Check sheet for the modelled part. Datum: model origin and axes. Units: mm. A direction names the side the tool comes from. Round coordinates to 2 decimals unless told otherwise and drop trailing zeros. Order: outer loops, then holes, each group sorted by start corner. A loop starts at its lowest first (then second) coordinate and runs counter-clockwise, first axis right, second up. Notation, with made-up numbers: (80, 67.25) -> (117, 67.25) arc R29 cw to (117, 106.25) -> close; hole circle Ø2 at (28.25, 60). An arc over 180 degrees is marked (long way). Answer in a Markdown table with one row per item. Add a question column.
1. Sectioned sample at B-B, the plane z = 0. Record the boundary of the cut face in (x, y) (3 decimals), then the cut area to 3 significant figures.
2. Sectioned sample at C-C, the plane y = 28. Record the boundary of the cut face in (x, z) (3 decimals).
3. Sectioned sample at A-A, the plane y = 3. Count the separate pieces of the cut face and the enclosed holes in it, then the cut area to 3 significant figures.
4. Access from +Z, -Z, +X, -X, +Y, -Y to the whole of each face (thin tool, end or side, straight path). Record for faces 1 (the flat face through (43.4, 11.768, -68.4)), 2 (the flat face through (76, 51.143, 0)), 3 (the flat face through (7.501, 57, 76)), 4 (the flat face through (-1, 11.768, -1)).
5. Material ranges on L1, parallel to Z at x = -6.5, y = 7.5; L2, parallel to X at y = 42.5, z = -4; L3, parallel to X at y = 58.5, z = -48, recorded low to high. Write a range as from..to.
6. Depth check by flat-ended pin: P1, Ø4.5, axis at y = 57, z = -76, coming from the -X side; P2, Ø5, axis at x = -1, z = -75.5, coming from the +Y side; P3, Ø6, axis at x = 37.5, y = 16, coming from the +Z side; P4, Ø9, axis at x = 0, z = 103.12, coming from the -Y side. Enter the tip coordinate at first touch or a pass-through.
7. Draft check along Z on faces 5 (the flat face through (0, 51.143, -76)), 6 (the flat face through (-76, 57, -7.5)), 7 (the cylindrical face through (30.881, 51.936, -74.477)), 8 (the flat face through (-76, 57, 7.5)). Enter one of: +Z half, -Z half, draft (parallel to the pull), parting line (faces both ways), or undercut.
```python
from build123d import *

# Parameters (mm, degrees)
SKETCH3_W          = 31.782249742
SKETCH3_H          = 8
SKETCH3_W_2        = 8
SKETCH3_H_2        = 31.782249742
CUT_EXTRUDE1_DEPTH = 6
CHAMFER1_SIZE      = 2
SKETCH4_R          = 4
CUT_EXTRUDE2_DEPTH = 67
SCALE_1_SCALE      = 1.875


with BuildPart() as part:
    # Sketch2 → Revolve1 (revolve)
    with BuildSketch(Plane.XY, mode=Mode.PRIVATE) as revolve1_sk:
        with BuildLine():
            Line((65, 9), (65, 0))
            Line((65, 0), (31, 0))
            Line((31, 0), (29, 2))
            Line((29, 2), (0, 2))
            Line((0, 2), (0, 11))
            Line((0, 11), (30.347168885, 11))
            ThreePointArc((30.347168885, 11), (33.667283917, 12.261439291), (35.312149528, 15.40926553))
            Line((35.312149528, 15.40926553), (39, 38))
            Line((39, 38), (43, 38))
            Line((43, 38), (43, 27))
            Line((43, 27), (45, 27))
            Line((45, 27), (45, 11))
            Line((45, 11), (43, 11))
            Line((43, 11), (43, 9))
            Line((43, 9), (65, 9))
        make_face()
    revolve(revolve1_sk.sketch.rotate(Axis((0, 2, 0), (0, 1, 0)), 90), axis=Axis((0, 2, 0), (0, 1, 0)))

    # Sketch3 → Cut-Extrude1 (cut)
    with BuildSketch(Plane(origin=(0, 38, 0), x_dir=(1, 0, 0), z_dir=(0, 1, 0))):
        with Locations((40.073271414, 0)):
            Rectangle(SKETCH3_W, SKETCH3_H)
        with Locations((0, 40.073271414)):
            Rectangle(SKETCH3_W_2, SKETCH3_H_2)
        with Locations((0, -40.073271414)):
            Rectangle(SKETCH3_W_2, SKETCH3_H_2)
        with Locations((-40.073271414, 0)):
            Rectangle(SKETCH3_W, SKETCH3_H)
    extrude(amount=-CUT_EXTRUDE1_DEPTH, mode=Mode.SUBTRACT)

    # Chamfer1
    chamfer1_edges = [part.edges().sort_by_distance(p)[0] for p in [
        (0, 0, 65),
    ]]
    chamfer(chamfer1_edges, length=CHAMFER1_SIZE)

    # Sketch4 → Cut-Extrude2 (cut)
    with BuildSketch(Plane(origin=(0, 38, 0), x_dir=(1, 0, 0), z_dir=(0, 1, 0))):
        with Locations(Location((0, 55, 0), (0, 0, 270))):
            Circle(SKETCH4_R)
        with Locations(Location((47.817664455, 27.174822282, 0), (0, 0, 270))):
            Circle(SKETCH4_R)
        with Locations(Location((-47.631397208, 27.5, 0), (0, 0, 270))):
            Circle(SKETCH4_R)
        with Locations(Location((-47.631397208, -27.5, 0), (0, 0, 270))):
            Circle(SKETCH4_R)
        with Locations(Location((0, -55, 0), (0, 0, 270))):
            Circle(SKETCH4_R)
        with Locations(Location((47.817664455, -27.174822282, 0), (0, 0, 270))):
            Circle(SKETCH4_R)
    extrude(amount=-CUT_EXTRUDE2_DEPTH, mode=Mode.SUBTRACT)


with BuildPart() as part_1:
    # Scale 1: scaled about (-0.000976977, 10.122102603, 0)
    add(part.part.scale(SCALE_1_SCALE).moved(Location((0.000854855, -8.856839778, 0))))


solid = part_1.part
```
Answer key:
| question | item | result |
|---|---|---|
| 1 | outline | (-121.874, -5.107) -> (-118.124, -8.857) -> (-58.124, -8.857) -> (-54.374, -5.107) -> (54.376, -5.107) -> (58.126, -8.857) -> (118.126, -8.857) -> (121.876, -5.107) -> (121.876, 8.018) -> (80.626, 8.018) -> (80.626, 11.768) -> (84.376, 11.768) -> (84.376, 41.768) -> (80.626, 41.768) -> (80.626, 51.143) -> (71.289, 51.143) -> (66.211, 20.036) arc R9.375 cw to (56.902, 11.768) -> (-56.9, 11.768) arc R9.375 cw to (-66.209, 20.036) -> (-71.288, 51.143) -> (-80.624, 51.143) -> (-80.624, 41.768) -> (-84.374, 41.768) -> (-84.374, 11.768) -> (-80.624, 11.768) -> (-80.624, 8.018) -> (-121.874, 8.018) -> close |
| 1 | area | 5,520 mm² |
| 2 | outline | circle Ø168.75 at (0.001, 0); hole circle Ø135.021 at (0.001, 0) |
| 3 | separate pieces | 1 |
| 3 | enclosed holes | 6 |
| 3 | area | 45,600 mm² |
| 4 | face 1 | none |
| 4 | face 2 | +X, -X, +Y |
| 4 | face 3 | +Z, -Z, +Y |
| 4 | face 4 | +Y |
| 5 | L1 | z = -121.7..-106.87, -99.38..99.38, 106.87..121.7 |
| 5 | L2 | x = -80.52..-69.76, 69.76..80.53 |
| 5 | L3 | x = -64.78..-54.32, 54.32..64.78 |
| 6 | P1 | stops at x = -32.58 |
| 6 | P2 | stops at y = 51.14 |
| 6 | P3 | stops at z = 77 |
| 6 | P4 | passes through |
| 7 | face 5 | draft |
| 7 | face 6 | undercut |
| 7 | face 7 | parting line |
| 7 | face 8 | undercut |
